```python
from build123d import *

# Parameters (mm, degrees)
CUT_EXTRUDE_1_DEPTH = 2.58


with BuildPart() as part:
    # 草图1 → 旋转1 (revolve)
    with BuildSketch(Plane.XY):
        with BuildLine():
            Line((0, 2), (-7.435105037, 2))
            ThreePointArc((-7.435105037, 2), (-7.513251262, 2.015899029), (-7.578972997, 2.061068326))
            Line((-7.578972997, 2.061068326), (-9.914908162, 4.48))
            Line((-9.914908162, 4.48), (-10, 4.48))
            Line((-10, 4.48), (-10, 0))
            Line((-10, 0), (0, 0))
            Line((0, 0), (0, 2))
        make_face()
    revolve(axis=Axis((0, 0, 0), (-1, 0, 0)))

    # 草图2 → 切除-拉伸1 (cut)
    with BuildSketch(Plane.ZY.offset(10)):
        Polygon((0, 1.443375673), (-1.25, 0.721687836), (-1.25, -0.721687836), (0, -1.443375673), (1.25, -0.721687836), (1.25, 0.721687836), align=None)
    extrude(amount=-CUT_EXTRUDE_1_DEPTH, mode=Mode.SUBTRACT)

    # 草图6 → 旋转2 (revolve)
    with BuildSketch(Plane.XY, mode=Mode.PRIVATE) as revolve_2_sk:
        Polygon((-8.5, 1.443375673), (-7.666666667, 0), (-7.05, 0), (-7.05, 1.443375673), align=None)
    revolve(revolve_2_sk.sketch.rotate(Axis((-10, 0, 0), (1, 0, 0)), 90), axis=Axis((-10, 0, 0), (1, 0, 0)))

    # 草图7 → 切除-旋转2 (revolve, cut)
    with BuildSketch(Plane.XY):
        Polygon((-10, 1.443375673), (-10, 0), (-9.593, 0), align=None)
    revolve(axis=Axis((-10, 0, 0), (1, 0, 0)), mode=Mode.SUBTRACT)

    # 草图4 → 切除-旋转1 (revolve, cut)
    with BuildSketch(Plane.XY):
        Polygon((-0.35, 2), (0, 1.393782217), (0.35, 2), align=None)
    revolve(axis=Axis((-0.35, 0, 0), (1, 0, 0)), mode=Mode.SUBTRACT)


solid = part.part
```
Here's how the part is built. I have some questions about the finished solid (model axes, mm). A direction names the side the tool comes from. Give positions to 0.01 mm unless a question says otherwise; leave off trailing zeros. Order: outer loops, then holes, each group sorted by start corner. A loop starts at its lowest first (then second) coordinate and runs counter-clockwise, first axis right, second up. Notation, with made-up numbers: M 88,-27.75 L 145,-27.75 A16 ccw 145,-14.75 Z; hole C -39,63 d11. An arc over 180 degrees is marked long. Use a Markdown table: item, result. Add a question column.
1. I need wall thicknesses on probe 1 along X at (y, z) = (-3, -0.25); probe 2 along X at (y, z) = (1.25, 0); probe 3 along Y at (x, z) = (-9, -1.75). Which ranges of each line are inside material? Lowest first, please. Write a range as from..to.
2. If we mould it in two halves opening along Z, with no side actions, what happens to faces 1 (the conical face through (-7.725, 1.021, 1.963)), 2 (the flat face through (-9.21, -1.08, -0.63)), 3 (the flat face through (0, 0, 0)), 4 (the flat face through (-9, 0, 1.25))? For each: +Z half, -Z half, draft (parallel to the pull), parting line (faces both ways), or undercut.
3. For pin 1 Ø3 at (x, z) = (-8, 2) entering from +Y; pin 2 Ø5 at (x, z) = (-6.5, 2) entering from +Y; pin 3 Ø4 at (x, y) = (-1.5, 0.5) entering from -Z; pin 4 Ø4 at (y, z) = (0, -1) entering from +X, each with a flat end and sliding along its axis, tell me the tip position at first contact or that it passes through.
4. Suppose I cut it at A-A (x = -4.5). List the corners of the cut face in (y, z) for me, and give its area (3 significant figures).
5. On a 3-axis mill with a long thin cutter (end or side, diameter ignored), from which of +Z, -Z, +X, -X, +Y, -Y can I reach the whole of each face in a straight line? I mean faces 5 (the flat face through (-9.205, 1.088, -0.616)), 6 (the cylindrical face through (-4, 0, 2)), 7 (the flat face through (-10, 2, 0)). Say none if no direction works.
Results list:
| question | item | result |
|---|---|---|
| 1 | probe 1 | x = -10..-8.5 |
| 1 | probe 2 | x = -8.39..0 |
| 1 | probe 3 | y = -3.07..3.07 |
| 2 | face 1 | parting line |
| 2 | face 2 | undercut |
| 2 | face 3 | draft |
| 2 | face 4 | undercut |
| 3 | pin 1 | stops at y = 3.67 |
| 3 | pin 2 | stops at y = 3.18 |
| 3 | pin 3 | stops at z = -2 |
| 3 | pin 4 | stops at x = 0 |
| 4 | outline | C 0,0 d4 |
| 4 | area | 12.6 mm² |
| 5 | face 5 | -X |
| 5 | face 6 | +X |
| 5 | face 7 | +Z, -Z, -X, +Y, -Y |
